Read the model definition and answer for the solid it produces. Units are mm, in the model's axes. A direction names the side the tool comes from. Give positions to 0.01 mm unless a question says otherwise; leave off trailing zeros. Order: outer loops, then holes, each group sorted by start corner. A loop starts at its lowest first (then second) coordinate and runs counter-clockwise, first axis right, second up. Notation, with made-up numbers: (14, 17) -> (69, 17) arc R36 ccw to (69, 56) -> close; hole circle Ø2 at (-38.75, 32). An arc over 180 degrees is marked (long way). Answer as CSV lines item,"result". Start each with the question number.
1) The mould has two halves that part along X. Classify faces 4 (the face through (0, 0, -9)), 5 (the face through (0.07, 20.98, 0.49)), 6 (the face through (16.7, -7.09, 1.49)), 7 (the face through (-18.206, -10.427, 0.493)): +X half, -X half, draft (parallel to the pull), parting line (faces both ways), or undercut.
2) Find section C-C (x = 0). Determine the outline of the cut face in (y, z).
3) Find section B-B (x = 5). Determine the outline of the cut face in (y, z), and give its area (3 significant figures).
4) For faces 1 (the face through (0, 0, 1)), 2 (the face through (-0.391, 18.955, -4.056)), 3 (the face through (-0.391, 18.955, -9.507)), determine the directions among +Z, -Z, +X, -X, +Y, -Y from which every point of the face is accessible in a straight line to the end or side of a thin tool.
5) Find section A-A (y = 5.5). Determine the outline of the cut face in (x, z).
6) Straight lines are drawn through the part: L1, parallel to Z at x = -14, y = -3; L2, parallel to X at y = 16, z = 1.25; L3, parallel to X at y = -10, z = -9.5. For each, find the intervals that lie inside material, in ascending order. Write a range as from..to.
7) Flat-ended cylindrical pins translate along their axes: pin 1 Ø10 at (x, y) = (8.5, 12.5) entering from -Z; pin 2 Ø1.5 at (y, z) = (0.5, 0) entering from +X; pin 3 Ø17 at (x, y) = (6, 5.5) entering from +Z. Find the tip coordinate at first contact, or state that the pin passes through.
8) Find section D-D (z = -3.5). Determine the outline of the cut face in (x, y).
```python
from build123d import *

# Parameters (mm, degrees)
SKETCH1_R           = 3
BOSS_EXTRUDE1_DEPTH = 1
BOSS_EXTRUDE2_START = -11
SKETCH2_R           = 3
BOSS_EXTRUDE2_DEPTH = 11
SKETCH3_R           = 3
BOSS_EXTRUDE3_DEPTH = 1


with BuildPart() as part:
    # Sketch1 → Boss-Extrude1 (new body)
    with BuildSketch(Plane.XY):
        with BuildLine():
            Line((18.169872981, -5.490381057), (4.330127019, 18.480762114))
            ThreePointArc((4.330127019, 18.480762114), (0, 20.980762114), (-4.330127019, 18.480762114))
            Line((-4.330127019, 18.480762114), (-18.169872981, -5.490381057))
            ThreePointArc((-18.169872981, -5.490381057), (-18.169872981, -10.490381057), (-13.839745962, -12.990381057))
            Line((-13.839745962, -12.990381057), (13.839745962, -12.990381057))
            ThreePointArc((13.839745962, -12.990381057), (18.169872981, -10.490381057), (18.169872981, -5.490381057))
        make_face()
        with Locations((0, 15.980762114)):
            Circle(SKETCH1_R, mode=Mode.SUBTRACT)
        with Locations((13.839745962, -7.990381057)):
            Circle(SKETCH1_R, mode=Mode.SUBTRACT)
        with Locations((-13.839745962, -7.990381057)):
            Circle(SKETCH1_R, mode=Mode.SUBTRACT)
    boss_extrude1 = extrude(amount=BOSS_EXTRUDE1_DEPTH)

    # Sketch2 → Boss-Extrude2 (add)
    with BuildSketch(Plane.XY.offset(1).offset(BOSS_EXTRUDE2_START)):
        with Locations((13.839745962, -7.990381057)):
            Circle(SKETCH2_R)
        with Locations((-13.839745962, -7.990381057)):
            Circle(SKETCH2_R)
        with Locations((0, 15.980762114)):
            Circle(SKETCH2_R)
    extrude(amount=BOSS_EXTRUDE2_DEPTH)

    # Mirror3: Boss-Extrude1 across plane
    add(boss_extrude1.mirror(Plane(origin=(0, 0, -4), x_dir=(1, 0, 0), z_dir=(0, 0, -1))))

    # Sketch3 → Boss-Extrude3 (add)
    with BuildSketch(Plane.XY.offset(1)):
        with Locations((0, 15.980762114)):
            Circle(SKETCH3_R)
        with Locations((13.839745962, -7.990381057)):
            Circle(SKETCH3_R)
        with Locations((-13.839745962, -7.990381057)):
            Circle(SKETCH3_R)
    extrude(amount=BOSS_EXTRUDE3_DEPTH)


solid = part.part
```
Findings below:
1,face 4,"undercut"
1,face 5,"parting line"
1,face 6,"undercut"
1,face 7,"-X half"
2,outline,"(-12.99, -9) -> (12.98, -9) -> (12.98, -10) -> (18.98, -10) -> (18.98, -9) -> (20.98, -9) -> (20.98, -8) -> (18.98, -8) -> (18.98, 0) -> (20.98, 0) -> (20.98, 1) -> (18.98, 1) -> (18.98, 2) -> (12.98, 2) -> (12.98, 1) -> (-12.99, 1) -> (-12.99, 0) -> (12.98, 0) -> (12.98, -8) -> (-12.99, -8) -> close"
3,outline,"(-12.99, -9) -> (17.32, -9) -> (17.32, -8) -> (-12.99, -8) -> close; (-12.99, 0) -> (17.32, 0) -> (17.32, 1) -> (-12.99, 1) -> close"
3,area,"60.6 mm²"
4,face 1,"+Z"
4,face 2,"none"
4,face 3,"-Z"
5,outline,"(-11.82, -9) -> (11.82, -9) -> (11.82, -8) -> (-11.82, -8) -> close; (-11.82, 0) -> (11.82, 0) -> (11.82, 1) -> (-11.82, 1) -> close"
6,L1,"-9..-8, 0..1"
6,L2,"-3..3"
6,L3,"-16.07..-11.61, 11.61..16.07"
7,pin 1,"z = -9"
7,pin 2,"x = 15.14"
7,pin 3,"z = 1"
8,outline,"circle Ø6 at (-13.84, -7.99); circle Ø6 at (0, 15.98); circle Ø6 at (13.84, -7.99)"
